Source: CAD feature listing. Evaluate the final solid. Frame: model axes, mm. Round coordinates to 2 decimals unless told otherwise and drop trailing zeros. Loops run counter-clockwise (first coordinate to the right, second up) from the corner with the lowest first, then second, coordinate; pieces in that order, holes last. Notation, with made-up numbers: M 71,66.5 L 97,66.5 A25 cw 97,88.5 Z; hole C 21,88.25 d8. An arc over 180 degrees is marked long. One line per item, written item: value.
from build123d import *

# Parameters (mm, degrees)
BOSS_EXTRUDE1_DEPTH = 20


with BuildPart() as part:
    # Sketch1 → Boss-Extrude1 (new body)
    with BuildSketch(Plane.XY):
        Polygon((7408.989913804, 2462.985883167), (7408.989913804, 4648.985876948), (7658.989913804, 4648.985876948), (7658.989913804, 2462.985883253), align=None)
        with BuildLine():
            Line((7508.989913506, 4367.985877479), (7558.989913353, 4367.985877479))
            ThreePointArc((7558.989913353, 4367.985877479), (7583.98991328, 4342.985877555), (7558.989913357, 4317.985877628))
            Line((7558.989913357, 4317.985877628), (7508.99011555, 4317.985877628))
            ThreePointArc((7508.99011555, 4317.985877628), (7483.989632688, 4342.98577653), (7508.989913506, 4367.985877479))
        make_face(mode=Mode.SUBTRACT)
        with BuildLine():
            Line((7508.990115362, 3087.985881301), (7558.98932559, 3087.985881301))
            ThreePointArc((7558.98932559, 3087.985881301), (7583.989619399, 3062.986175259), (7558.989913357, 3037.98588145))
            Line((7558.989913357, 3037.98588145), (7508.989913506, 3037.98588145))
            ThreePointArc((7508.989913506, 3037.98588145), (7483.989913645, 3062.985982304), (7508.990115362, 3087.985881301))
        make_face(mode=Mode.SUBTRACT)
        with BuildLine():
            Line((7508.989913506, 4067.985878375), (7558.989913353, 4067.985878375))
            ThreePointArc((7558.989913353, 4067.985878375), (7583.989913278, 4042.985878449), (7558.989913353, 4017.985878524))
            Line((7558.989913353, 4017.985878524), (7508.990115553, 4017.985878524))
            ThreePointArc((7508.990115553, 4017.985878524), (7483.989632674, 4042.985777424), (7508.989913506, 4067.985878375))
        make_face(mode=Mode.SUBTRACT)
        with BuildLine():
            Line((7508.989913506, 2787.985882197), (7558.989325591, 2787.985882197))
            ThreePointArc((7558.989325591, 2787.985882197), (7583.989619399, 2762.986176154), (7558.989913357, 2737.985882346))
            Line((7558.989913357, 2737.985882346), (7508.989913506, 2737.985882346))
            ThreePointArc((7508.989913506, 2737.985882346), (7483.989770854, 2762.985882271), (7508.989913506, 2787.985882197))
        make_face(mode=Mode.SUBTRACT)
    extrude(amount=BOSS_EXTRUDE1_DEPTH)


solid = part.part
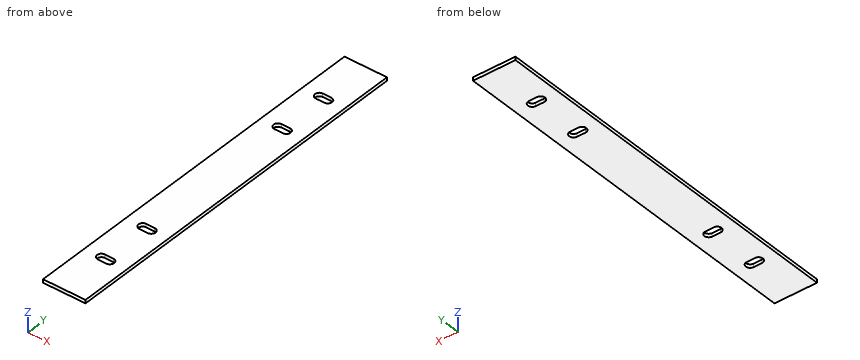
1. Section query A-A (z = 3.75). Return the cut outline in (x, y), and give its area (3 significant figures).
Report:
outline: M 7408.99,2462.99 L 7658.99,2462.99 L 7658.99,4648.99 L 7408.99,4648.99 Z; hole M 7508.99,2737.99 L 7558.99,2737.99 A25 ccw 7558.99,2787.99 L 7508.99,2787.99 A25 ccw Z; hole M 7508.99,3037.99 L 7558.99,3037.99 A25 ccw 7558.99,3087.99 L 7508.99,3087.99 A25 ccw Z; hole M 7508.99,4017.99 L 7558.99,4017.99 A25 ccw 7558.99,4067.99 L 7508.99,4067.99 A25 ccw Z; hole M 7508.99,4317.99 L 7558.99,4317.99 A25 ccw 7558.99,4367.99 L 7508.99,4367.99 A25 ccw Z
area: 529,000 mm2
2. Ray query, line 1 (Y direction, x = 7546, z = 7.75); line 2 (Y direction, x = 7563.5, z = 14.75); line 3 (X direction, y = 4054.5, z = 9). Return the intervals inside material, ascending. Write a range as [from, to].
Report:
line 1: y = [2462.99, 2737.99], [2787.99, 3037.99], [3087.99, 4017.99], [4067.99, 4317.99], [4367.99, 4648.99]
line 2: y = [2462.99, 2738.4], [2787.58, 3038.4], [3087.58, 4018.4], [4067.58, 4318.4], [4367.58, 4648.99]
line 3: x = [7408.99, 7486.8], [7581.18, 7658.99]
3. Pin query (flat end, axial travel): pin 1 (6 mm diameter, centred on x = 7498, y = 3857, fed in from -Z). Return the tip coordinate at first contact, or that it passes through.
Report:
pin 1: stops at z = 0
